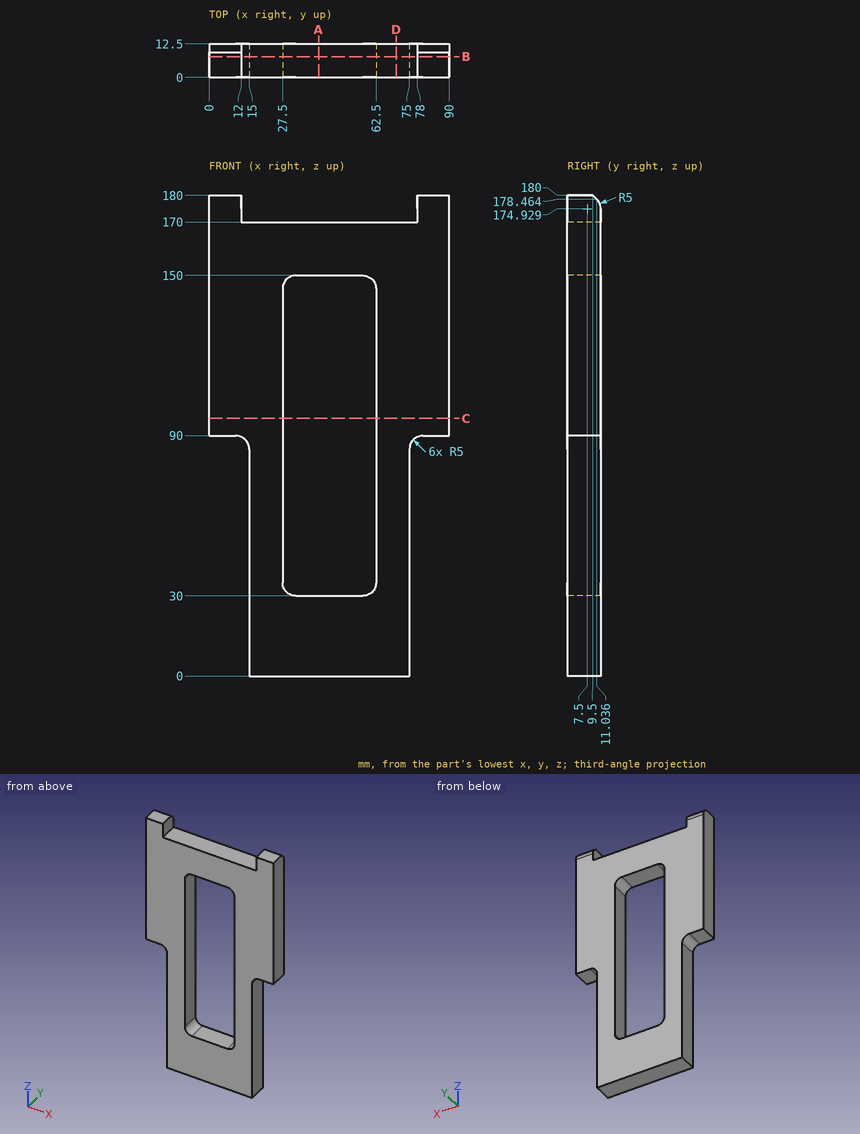
Here's the drawing with two shaded views (mm, measured from the low corner). I have some questions. Coordinates: 2 decimals unless noted, no trailing zeros. Order: outer loops, then holes, each group sorted by start corner. A loop starts at its lowest first (then second) coordinate and runs counter-clockwise, first axis right, second up. Notation, with made-up numbers: (-13.75, 20) -> (8.25, 20) arc R8 ccw to (8.25, 24) -> close; hole circle Ø1 at (6, -24). An arc over 180 degrees is marked (long way). One line per question, with ' | ' between items.
Q1. Imagine slicing it at D-D on x = 70. Please give me the cut outline in (y, z), and give its area (4 significant figures).
Return value:
outline: (0, 0) -> (12.5, 0) -> (12.5, 170) -> (0, 170) -> close | area: 2,125 mm²
Q2. I'm going to push flat-ended pins straight in: P1, Ø4, axis at x = 45.5, y = 5, coming from the +Z side; P2, Ø2, axis at y = 10.5, z = 26.5, coming from the +X side; P3, Ø5, axis at x = 5.5, y = 6, coming from the -Z side. Where does each tip first touch, or does it pass through?
Return value:
P1: z = 170 | P2: x = 75 | P3: z = 90
Q3. If I drill on L1, parallel to X at y = 7, z = 144; L2, parallel to X at y = 11.5, z = 82; L3, parallel to Z at x = 39, y = 1.25, over which ranges is the centre line in solid material (lowest first)?
Return value:
L1: 0 to 27.5, 62.5 to 90 | L2: 15 to 27.5, 62.5 to 75 | L3: 0 to 30, 150 to 170
Q4. Imagine slicing it at B-B on y = 7.75. Please give me the cut outline in (x, z), and give its area (3 significant figures).
Return value:
outline: (0, 90) -> (10, 90) arc R5 cw to (15, 85) -> (15, 0) -> (75, 0) -> (75, 85) arc R5 cw to (80, 90) -> (90, 90) -> (90, 180) -> (78, 180) -> (78, 170) -> (12, 170) -> (12, 180) -> (0, 180) -> close; hole (27.5, 35) arc R5 ccw to (32.5, 30) -> (57.5, 30) arc R5 ccw to (62.5, 35) -> (62.5, 145) arc R5 ccw to (57.5, 150) -> (32.5, 150) arc R5 ccw to (27.5, 145) -> close | area: 8,670 mm²
Q5. Imagine slicing it at C-C on z = 96.5. Please give me the cut outline in (x, y).
Return value:
outline: (0, 0) -> (27.5, 0) -> (27.5, 12.5) -> (0, 12.5) -> close; (62.5, 0) -> (90, 0) -> (90, 12.5) -> (62.5, 12.5) -> close
Q6. Imagine slicing it at A-A on x = 41. Please give me the cut outline in (y, z).
Return value:
outline: (0, 0) -> (12.5, 0) -> (12.5, 30) -> (0, 30) -> close; (0, 150) -> (12.5, 150) -> (12.5, 170) -> (0, 170) -> close
